Build history of the part. All positions in model axes, mm. Face numbers are marked on the shaded views. Give positions to 0.01 mm unless a question says otherwise; leave off trailing zeros. Loops run counter-clockwise (first coordinate to the right, second up) from the corner with the lowest first, then second, coordinate; pieces in that order, holes last. Notation, with made-up numbers: M -34,44 L 17,44 A24 cw 17,78 Z; hole C -12,-2 d7. An arc over 180 degrees is marked long. Put each result on its own line as item: value.
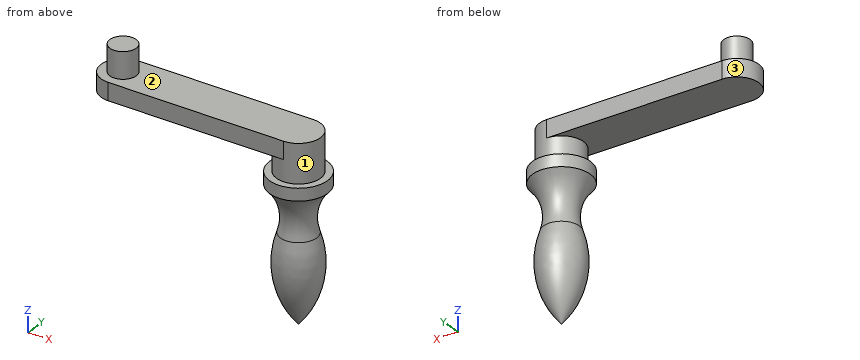
```python
from build123d import *

# Parameters (mm, degrees)
EXTRUDE_1_DEPTH = 10
SKETCH_2_R      = 7.5
EXTRUDE_2_DEPTH = 15


with BuildPart() as part:
    # 草图1 → 凸台-拉伸1 (new body)
    with BuildSketch(Plane.XY):
        with BuildLine():
            Line((0, 0), (100, 0))
            ThreePointArc((100, 0), (112.5, 12.5), (100, 25))
            Line((100, 25), (0, 25))
            ThreePointArc((0, 25), (-12.5, 12.5), (0, 0))
        make_face()
    extrude(amount=EXTRUDE_1_DEPTH)

    # 草图2 → 凸台-拉伸2 (add)
    with BuildSketch(Plane.XY.offset(10)):
        with Locations((0, 12.5)):
            Circle(SKETCH_2_R)
    extrude(amount=EXTRUDE_2_DEPTH)

    # 草图7 → 旋转1 (revolve)
    with BuildSketch(Plane(origin=(100, 0, 0), x_dir=(0, 0, -1), z_dir=(1, 0, 0)), mode=Mode.PRIVATE) as revolve_1_sk:
        with BuildLine():
            Line((0, 12.5), (0, 25))
            Line((0, 25), (12, 25))
            Line((12, 25), (12, 29))
            Line((12, 29), (19, 29))
            ThreePointArc((19, 29), (31.116731463, 22.12336259), (45.032630645, 22.794982573))
            ThreePointArc((45.032630645, 22.794982573), (71.367513527, 24.466816677), (94.885940011, 12.5))
            Line((94.885940011, 12.5), (0, 12.5))
        make_face()
    revolve(revolve_1_sk.sketch.rotate(Axis((100, 12.5, 0), (0, 0, -1)), 180), axis=Axis((100, 12.5, 0), (0, 0, -1)))


solid = part.part
```
Q1. Probe line 1 (Z direction, x = 77.5, y = 8); line 2 (Z direction, x = -2.5, y = 6.5). List the from-to ranges inside material, lowest first. Write a range as from..to.
Here are the results:
line 1: 0..10
line 2: 0..25
Q2. Drop flat-ended pins along their axis: pin 1 Ø12 at (x, y) = (85, 5) entering from +Z; pin 2 Ø3 at (y, z) = (4, -24.5) entering from -X; pin 3 Ø3 at (x, y) = (40.5, 21.5) entering from -Z. Give the stop position or say it passes through.
Here are the results:
pin 1: z = 10
pin 2: x = 89.48
pin 3: z = 0
Q3. Slice it at B-B (z = -15). List the corners of the cut face in (x, y).
Here are the results:
outline: C 100,12.5 d33
Q4. Slice it at A-A (x = 3). List the corners of the cut face in (y, z).
Here are the results:
outline: M 0,0 L 25,0 L 25,10 L 19.37,10 L 19.37,25 L 5.63,25 L 5.63,10 L 0,10 Z
Q5. Slice it at C-C (x = 54). List the corners of the cut face in (y, z).
Here are the results:
outline: M 0,0 L 25,0 L 25,10 L 0,10 Z
Q6. Mould opens along Z. For the marked faces 1, 2 and 3 say: pulls with the +Z half, pulls with the -Z half, needs draft (parallel to the pull), parting line crosses it, or undercut.
Here are the results:
face 1: undercut
face 2: pulls with the +Z half
face 3: needs draft
